Geometry: final body of the model. Coordinates: model frame, mm. A direction names the side the tool comes from. Give positions to 0.01 mm unless a question says otherwise; leave off trailing zeros. Write each loop counter-clockwise with the first axis right and the second up, starting at its lowest first coordinate (ties: lowest second). Pieces come first, ordered by that corner, then holes. Notation, with made-up numbers: M 71.5,42.25 L 84.5,42.25 A18 cw 84.5,56.25 Z; hole C 4,8 d1. An arc over 180 degrees is marked long. Answer as a JSON object with one key per item and string values.
from build123d import *

# Parameters (mm, degrees)
EXTRUDE_1_DEPTH           = 30
HOLE_WIZARD_1_D           = 3.4
HOLE_WIZARD_1_CBORE_D     = 6
HOLE_WIZARD_1_CBORE_DEPTH = 3.4
PATTERN_LINEAR_1_COUNT    = 2
PATTERN_LINEAR_1_PITCH    = 40


with BuildPart() as part:
    # 草图2 → 凸台-拉伸1 (new, symmetric)
    with BuildSketch(Plane.XY):
        with BuildLine():
            Line((7.5, 9.7), (7.2, 10))
            Line((7.2, 10), (-7.2, 10))
            Line((-7.2, 10), (-7.5, 9.7))
            Line((-7.5, 9.7), (-7.5, 8.120037878))
            ThreePointArc((-7.5, 8.120037878), (-6.914137517, 7.982905386), (-6.45, 7.6))
            Line((-6.45, 7.6), (-5.6, 7.6))
            ThreePointArc((-5.6, 7.6), (-5.458578644, 7.541421356), (-5.4, 7.4))
            Line((-5.4, 7.4), (-5.4, 6.2))
            ThreePointArc((-5.4, 6.2), (-5.458578644, 6.058578644), (-5.6, 6))
            Line((-5.6, 6), (-6.45, 6))
            ThreePointArc((-6.45, 6), (-6.914137517, 5.617094614), (-7.5, 5.479962122))
            Line((-7.5, 5.479962122), (-7.5, 0.3))
            Line((-7.5, 0.3), (-7.2, 0))
            Line((-7.2, 0), (7.2, 0))
            Line((7.2, 0), (7.5, 0.3))
            Line((7.5, 0.3), (7.5, 5.479962122))
            ThreePointArc((7.5, 5.479962122), (6.914137517, 5.617094614), (6.45, 6))
            Line((6.45, 6), (5.6, 6))
            ThreePointArc((5.6, 6), (5.458578644, 6.058578644), (5.4, 6.2))
            Line((5.4, 6.2), (5.4, 7.4))
            ThreePointArc((5.4, 7.4), (5.458578644, 7.541421356), (5.6, 7.6))
            Line((5.6, 7.6), (6.45, 7.6))
            ThreePointArc((6.45, 7.6), (6.914137517, 7.982905386), (7.5, 8.120037878))
            Line((7.5, 8.120037878), (7.5, 9.7))
        make_face()
    extrude(amount=EXTRUDE_1_DEPTH, both=True)

    # 打孔尺寸(%根据)内六角圆柱头螺钉的类型1 (through all)
    with Locations(Plane(origin=(0, 10, 20), x_dir=(0, 0, 1), z_dir=(0, 1, 0))):
        with Locations((0, 0)):
            hole_wizard_1 = CounterBoreHole(HOLE_WIZARD_1_D / 2, HOLE_WIZARD_1_CBORE_D / 2, HOLE_WIZARD_1_CBORE_DEPTH)

    # 阵列(线性)1: 打孔尺寸(%根据)内六角圆柱头螺钉的类型1 ×2
    with Locations(*[(0, 0, -i * PATTERN_LINEAR_1_PITCH) for i in range(1, PATTERN_LINEAR_1_COUNT)]):
        add(hole_wizard_1, mode=Mode.SUBTRACT)


solid = part.part
1) Set-up query: faces 1 (the flat face through (-5.4, 7, 0)), 2 (the flat face through (5.4, 7, 0)), 3 (the flat face through (-2, 6.6, -20)). Return all of +Z, -Z, +X, -X, +Y, -Y with unobstructed straight access to the full face (end or side cutting, diameter ignored); none if empty.
Geometry check:
{"face 1": "+Z, -Z, -X", "face 2": "+Z, -Z, +X", "face 3": "+Y"}
2) Line query: line 1 (X direction, y = 9.15, z = 20); line 2 (X direction, y = 5, z = -20); line 3 (Z direction, x = -1.5, y = 1.5). Output: solid intervals per line, ascending. Write a range as from..to.
Geometry check:
{"line 1": "x = -7.5..-3, 3..7.5", "line 2": "x = -7.5..-1.7, 1.7..7.5", "line 3": "z = -30..-20.8, -19.2..19.2, 20.8..30"}
3) Pull-direction query (Z, two-part tool) for faces 4 (the flat face through (7.5, 3, 0)), 5 (the flat face through (-2, 6.6, 20)), 6 (the flat face through (0, 5, 30)), 7 (the flat face through (0, 5, -30)); classes: pulls with the +Z half, pulls with the -Z half, needs draft (parallel to the pull), parting line crosses it, or undercut.
Geometry check:
{"face 4": "needs draft", "face 5": "undercut", "face 6": "pulls with the +Z half", "face 7": "pulls with the -Z half"}
4) Cut plane B-B on x = 0. Return loops of the section in (y, z).
Geometry check:
{"outline": "M 0,-30 L 10,-30 L 10,-23 L 6.6,-23 L 6.6,-21.7 L 0,-21.7 Z; M 0,-18.3 L 6.6,-18.3 L 6.6,-17 L 10,-17 L 10,17 L 6.6,17 L 6.6,18.3 L 0,18.3 Z; M 0,21.7 L 6.6,21.7 L 6.6,23 L 10,23 L 10,30 L 0,30 Z"}
5) Cut plane C-C on z = -2.5. Return loops of the section in (x, y).
Geometry check:
{"outline": "M -7.5,0.3 L -7.2,0 L 7.2,0 L 7.5,0.3 L 7.5,5.48 A1.32 cw 6.45,6 L 5.6,6 A0.2 cw 5.4,6.2 L 5.4,7.4 A0.2 cw 5.6,7.6 L 6.45,7.6 A1.32 cw 7.5,8.12 L 7.5,9.7 L 7.2,10 L -7.2,10 L -7.5,9.7 L -7.5,8.12 A1.32 cw -6.45,7.6 L -5.6,7.6 A0.2 cw -5.4,7.4 L -5.4,6.2 A0.2 cw -5.6,6 L -6.45,6 A1.32 cw -7.5,5.48 Z"}
6) Contact query for flat-ended pins moving along their axis: P1, Ø5.5, axis at x = 0, z = 20, coming from the +Y side; P2, Ø0.6, axis at y = 7, z = -7, coming from the -X side. Output: stop coordinate, or through.
Geometry check:
{"P1": "stops at y = 6.6", "P2": "stops at x = -5.4"}
7) Cut plane D-D on y = 3. Return loops of the section in (x, z), and give its area (3 significant figures).
Geometry check:
{"outline": "M -7.5,-30 L 7.5,-30 L 7.5,30 L -7.5,30 Z; hole C 0,-20 d3.4; hole C 0,20 d3.4", "area": "882 mm2"}
